Design review of the part built by this model. Coordinates are the model's own, in mm. Face numbers are marked on the shaded views. Coordinates: 2 decimals unless noted, no trailing zeros. Write each loop counter-clockwise with the first axis right and the second up, starting at its lowest first coordinate (ties: lowest second). Pieces come first, ordered by that corner, then holes. Notation, with made-up numbers: (-18, -4.75) - (-9, -4.75) arc R15 cw to (-9, 6.25) - close; hole circle Ø11 at (-13.5, 85). An arc over 180 degrees is marked (long way). Use a Markdown table: item, result.
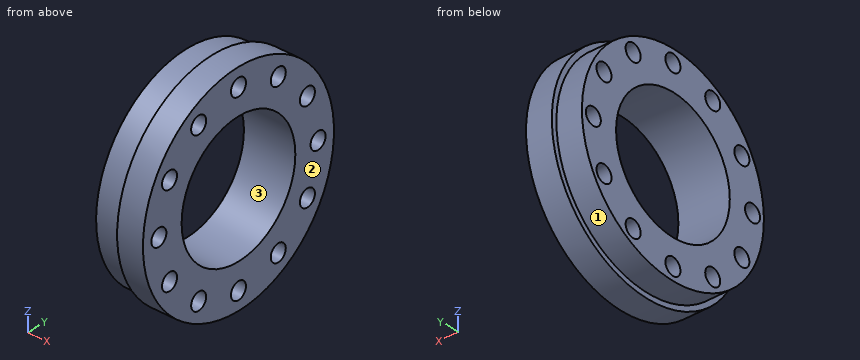
from build123d import *

# Parameters (mm, degrees)
HOLE_WIZARD_M4_1_D = 3.3


with BuildPart() as part:
    # 草图1 → 旋转1 (revolve)
    with BuildSketch(Plane(origin=(0, 0, 0), x_dir=(1, 0, 0), z_dir=(0, 1, 0)), mode=Mode.PRIVATE) as revolve_1_sk:
        Polygon((0, 12.5), (0, 20), (4.95, 20), (4.95, 21), (9.95, 21), (9.95, 12.5), align=None)
    revolve(revolve_1_sk.sketch.rotate(Axis((-63.943599205, 0, 0), (1, 0, 0)), 180), axis=Axis((-63.943599205, 0, 0), (1, 0, 0)))

    # M4 螺纹孔1 (through all)
    with Locations(Plane(origin=(9.95, 0, 0), x_dir=(0, 0, -1), z_dir=(1, 0, 0))):
        with Locations((0, 0), (0, 17.5), (8.75, 15.155444566), (15.155444566, 8.75), (17.5, 0), (15.155444566, -8.75), (8.75, -15.155444566), (0, -17.5), (-8.75, -15.155444566), (-15.155444566, -8.75), (-17.5, 0), (-15.155444566, 8.75), (-8.75, 15.155444566)):
            Hole(HOLE_WIZARD_M4_1_D / 2)


solid = part.part
(1) Draft analysis for pull direction Z (two halves, no side actions). For the marked faces 1, 2 and 3, state which applies: +Z half, -Z half, draft (parallel to the pull), parting line (faces both ways), or undercut.
Determined:
| item | result |
|---|---|
| face 1 | parting line |
| face 2 | draft |
| face 3 | undercut |
(2) Take a section at C-C on x = 6. State how many separate pieces and enclosed holes the cut face has, and give its area (3 significant figures).
Determined:
| item | result |
|---|---|
| separate pieces | 1 |
| enclosed holes | 13 |
| area | 792 mm2 |
(3) Take a section at D-D on z = 17.5. Write out the cut boundary in (x, y).
Determined:
| item | result |
|---|---|
| outline | (0, -9.68) - (4.95, -9.68) - (4.95, -11.61) - (9.95, -11.61) - (9.95, -1.65) - (0, -1.65) - close; (0, 1.65) - (9.95, 1.65) - (9.95, 11.61) - (4.95, 11.61) - (4.95, 9.68) - (0, 9.68) - close |
(4) For L1, parallel to Y at x = 8, z = 0; L2, parallel to Y at x = 3.25, z = 8.75; L3, parallel to Z at x = 1.5, y = 1.5, list the stretches that pass through material, from the lowest coordinate up. Write a range as from..to.
Determined:
| item | result |
|---|---|
| L1 | -21..-19.15, -15.85..-12.5, 12.5..15.85, 19.15..21 |
| L2 | -17.98..-16.81, -13.51..-8.93, 8.93..13.51, 16.81..17.98 |
| L3 | -19.94..-18.19, -16.81..-12.41, 12.41..16.81, 18.19..19.94 |
(5) Take a section at B-B on y = 6.5. Write out the cut boundary in (x, z), and give its area (3 significant figures).
Determined:
| item | result |
|---|---|
| outline | (0, -18.91) - (4.95, -18.91) - (4.95, -19.97) - (9.95, -19.97) - (9.95, -10.68) - (0, -10.68) - close; (0, 10.68) - (9.95, 10.68) - (9.95, 19.97) - (4.95, 19.97) - (4.95, 18.91) - (0, 18.91) - close |
| area | 174 mm2 |
(6) Take a section at A-A on z = 0. Write out the cut boundary in (x, y), and give its area (3 significant figures).
Determined:
| item | result |
|---|---|
| outline | (0, -20) - (4.95, -20) - (4.95, -21) - (9.95, -21) - (9.95, -19.15) - (0, -19.15) - close; (0, -15.85) - (9.95, -15.85) - (9.95, -12.5) - (0, -12.5) - close; (0, 12.5) - (9.95, 12.5) - (9.95, 15.85) - (0, 15.85) - close; (0, 19.15) - (9.95, 19.15) - (9.95, 21) - (4.95, 21) - (4.95, 20) - (0, 20) - close |
| area | 93.6 mm2 |
(7) For pin 1 (2 mm diameter, centred on y = 17.5, z = 0, fed in from -X); pin 2 (1 mm diameter, centred on x = 8, z = 1.5, fed in from -Y); pin 3 (5 mm diameter, centred on x = 2, y = 11, fed in from +Z); pin 4 (4 mm diameter, centred on x = 3.5, z = 9.5, fed in from -Y), all flat-tipped, find the tip position at first contact; note any pin that passes through.
Determined:
| item | result |
|---|---|
| pin 1 | through |
| pin 2 | y = -20.98 |
| pin 3 | z = 18.1 |
| pin 4 | y = -19.37 |
